Part model, mm, in its own coordinate system. Face numbers are marked on the shaded views. Coordinates: 2 decimals unless noted, no trailing zeros.
1) Wall check: L1, parallel to Z at x = -82.5, y = 48.5; L2, parallel to X at y = 52.5, z = -3; L3, parallel to X at y = 50.75, z = -5.75. Give the ranges that are in metal, low to high.
2) Mould opens along Y. For the marked faces 1, 2 and 3 say: +Y half, -Y half, draft (parallel to the pull), parting line (faces both ways), or undercut.
3) Pin check, flat tips, straight feed: pin 1 Ø1 at (y, z) = (48, 1) entering from -X; pin 2 Ø4 at (y, z) = (48.5, 2.5) entering from -X; pin 3 Ø1 at (x, y) = (-87, 51.5) entering from -Z. Stop position of each tip, or through.
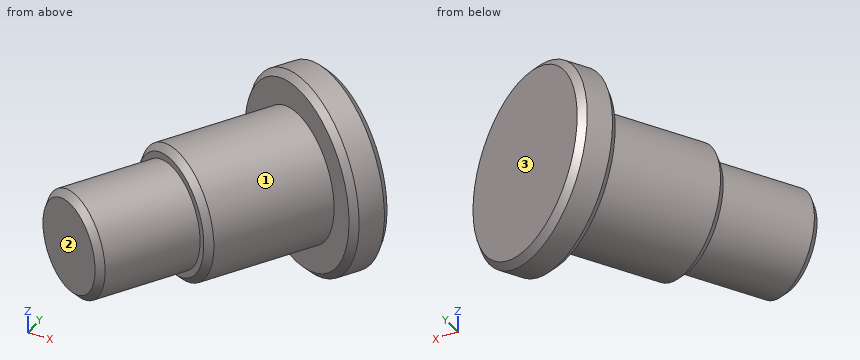
```python
from build123d import *

# Parameters (mm, degrees)
CHAMFER1_SIZE = 0.5


with BuildPart() as part:
    # Sketch1 → Revolve1 (revolve)
    with BuildSketch(Plane.XY, mode=Mode.PRIVATE) as revolve1_sk:
        Polygon((-80.994872981, 46.440861912), (-78.829809472, 45.190861912), (-77.329809472, 47.788938123), (-83.825, 51.538938123), (-94.325, 33.352404644), (-90.860898385, 31.352404644), (-86.860898385, 38.280607874), (-85.994872981, 37.780607874), align=None)
    revolve(revolve1_sk.sketch.rotate(Axis((-83.825, 51.538938123, 0), (-0.499999999999998, -0.8660254037844399, 0)), 180), axis=Axis((-83.825, 51.538938123, 0), (-0.499999999999998, -0.8660254037844399, 0)))

    # Chamfer1
    chamfer1_edges = [part.edges().sort_by_distance(p)[0] for p in [
        (-85.994872981, 37.780607874, 0),
        (-90.860898385, 31.352404644, 0),
        (-77.329809472, 47.788938123, 0),
        (-78.829809472, 45.190861912, 0),
    ]]
    chamfer(chamfer1_edges, length=CHAMFER1_SIZE)


solid = part.part
```
Geometry check:
1. L1: z = -7.01 to 7.01
1. L2: x = -90.93 to -85.49
1. L3: x = -88.46 to -82.46
2. face 1: undercut
2. face 2: -Y half
2. face 3: +Y half
3. pin 1: stops at x = -91.83
3. pin 2: stops at x = -92.09
3. pin 3: stops at z = -7.16
